from build123d import *

# Parameters (mm, degrees)
SKETCH1_W            = 80
SKETCH1_H            = 155
BOSS_EXTRUDE1_DEPTH  = 3
M4_TAPPED_HOLE1_D    = 3.3
M4_CLEARANCE_HOLE1_D = 4.5
SKETCH8_W            = 48
SKETCH8_H            = 65
CUT_EXTRUDE1_DEPTH   = 175.453432182
CHAMFER1_SIZE        = 3
FILLET1_R            = 10


with BuildPart() as part:
    # Sketch1 → Boss-Extrude1 (new body)
    with BuildSketch(Plane.XY):
        with Locations((40, 77.5)):
            Rectangle(SKETCH1_W, SKETCH1_H)
    extrude(amount=BOSS_EXTRUDE1_DEPTH)

    # M4 Tapped Hole1 (through all)
    with Locations(Plane.XY.offset(3)):
        with Locations((64, 82.5), (64, 7.5)):
            Hole(M4_TAPPED_HOLE1_D / 2)

    # M4 Clearance Hole1 (through all)
    with Locations(Plane.XY.offset(3)):
        with Locations((10, 82.5), (10, 7.5)):
            Hole(M4_CLEARANCE_HOLE1_D / 2)

    # Sketch8 → Cut-Extrude1 (cut, through all)
    with BuildSketch(Plane.XY.offset(3)):
        with Locations((24, 122.5)):
            Rectangle(SKETCH8_W, SKETCH8_H)
    extrude(amount=-CUT_EXTRUDE1_DEPTH, mode=Mode.SUBTRACT)

    # Chamfer1
    chamfer1_edges = [part.edges().sort_by_distance(p)[0] for p in [
        (48, 155, 1.5),
        (0, 90, 1.5),
        (80, 155, 1.5),
        (80, 0, 1.5),
        (0, 0, 1.5),
    ]]
    chamfer(chamfer1_edges, length=CHAMFER1_SIZE)

    # Fillet1
    fillet1_edges = [part.edges().sort_by_distance(p)[0] for p in [
        (48, 90, 1.5),
    ]]
    fillet(fillet1_edges, radius=FILLET1_R)


solid = part.part
Source: CAD feature listing. Evaluate the final solid. Frame: model axes, mm. A direction names the side the tool comes from. Give positions to 0.01 mm unless a question says otherwise; leave off trailing zeros. Write each loop counter-clockwise with the first axis right and the second up, starting at its lowest first coordinate (ties: lowest second). Pieces come first, ordered by that corner, then holes. Notation, with made-up numbers: M -23,-3 L 15,-3 A33 cw 15,26 Z; hole C 83,-21 d10. An arc over 180 degrees is marked long. Return JSON: item names as keys, results as strings. Group by question number.
1) Cut plane D-D, the plane y = 108.5. Output: boundary loops of the cut face in (x, z), then the cut area to 3 significant figures.
2) Cut plane C-C, the plane y = 82.5. Output: boundary loops of the cut face in (x, z), then the cut area to 3 significant figures.
3) Set-up query: faces 1 (the face through (0, 44, 1)), 2 (the face through (48, 126, 2)). Return all of +Z, -Z, +X, -X, +Y, -Y with unobstructed straight access to the full face (end or side cutting, diameter ignored); none if empty.
4) Cut plane B-B, the plane x = 10. Output: boundary loops of the cut face in (y, z).
5) Cut plane A-A, the plane z = 1.4. Output: boundary loops of the cut face in (x, y).
6) Ray query, L1, parallel to Y at x = 64, z = 0.95; L2, parallel to Y at x = 10, z = 1.15; L3, parallel to X at y = 128.5, z = 2.45. Return the intervals inside material, ascending.
7) First-contact query: pin 1 Ø1.5 at (y, z) = (100, 2) entering from -X; pin 2 Ø1.5 at (x, z) = (21.5, 1.5) entering from +Y. Flat tips, straight axial feed; report the tip coordinate or a pass-through.
8) Draft query along X for faces 3 (the face through (65.216, 8.615, 1.479)), 4 (the face through (2, 1, 1)), 5 (the face through (48, 61, 3)). Return one class per face: released by +X, released by -X, zero draft, split by the parting line, or undercut.
Data:
{
 "1": {"outline": "M 48,0 L 80,0 L 80,3 L 48,3 Z", "area": "96.0 mm²"},
 "2": {"outline": "M 0,0 L 7.75,0 L 7.75,3 L 0,3 Z; M 12.25,0 L 62.35,0 L 62.35,3 L 12.25,3 Z; M 65.65,0 L 80,0 L 80,3 L 65.65,3 Z", "area": "217 mm²"},
 "3": {"face 1": "+Z, -Z, -X, +Y, -Y", "face 2": "+Z, -Z, -X, +Y"},
 "4": {"outline": "M 0,0 L 5.25,0 L 5.25,3 L 0,3 Z; M 9.75,0 L 80.25,0 L 80.25,3 L 9.75,3 Z; M 84.75,0 L 90,0 L 90,3 L 84.75,3 Z"},
 "5": {"outline": "M 0,3 L 3,0 L 77,0 L 80,3 L 80,152 L 77,155 L 51,155 L 48,152 L 48,100 A10 cw 38,90 L 3,90 L 0,87 Z; hole C 10,7.5 d4.5; hole C 10,82.5 d4.5; hole C 64,7.5 d3.3; hole C 64,82.5 d3.3"},
 "6": {"L1": "y = 0 to 5.85, 9.15 to 80.85, 84.15 to 155", "L2": "y = 0 to 5.25, 9.75 to 80.25, 84.75 to 90", "L3": "x = 48 to 80"},
 "7": {"pin 1": "stops at x = 47.97", "pin 2": "stops at y = 90"},
 "8": {"face 3": "undercut", "face 4": "released by -X", "face 5": "zero draft"}
}
